from build123d import *

# Parameters (mm, degrees)
SWEEP1_PROFILE_R = 5


with BuildPart() as part:
    # Sweep1: sweep along a path in Sketch1
    with BuildLine(Plane.XY) as sweep1_path:
        Line((-60, 40), (-60, 10))
        ThreePointArc((-60, 10), (-57.071067812, 2.928932188), (-50, 0))
        Line((-50, 0), (50, 0))
        ThreePointArc((50, 0), (57.071067812, 2.928932188), (60, 10))
        Line((60, 10), (60, 40))
    # Sweep1 profile (on start of the path) → Sweep1 (sweep)
    with BuildSketch(Plane(origin=(-60, 40, 0), x_dir=(-1, 0, 0), z_dir=(0, -1, 0))):
        Circle(SWEEP1_PROFILE_R)
    sweep(path=sweep1_path.line)


solid = part.part
CAD build for the part. Positions are in the model's coordinates, mm. A direction names the side the tool comes from. Round coordinates to 2 decimals unless told otherwise and drop trailing zeros. Order: outer loops, then holes, each group sorted by start corner. A loop starts at its lowest first (then second) coordinate and runs counter-clockwise, first axis right, second up. Notation, with made-up numbers: (-1, 22.5) -> (26, 22.5) arc R31 cw to (26, 48.5) -> close; hole circle Ø4 at (86.5, 46.5). An arc over 180 degrees is marked (long way). Write item = value, one per line. Start each with the question number.
(1) Cut at B-B, the plane y = 31. List the corners of the cut face in (x, z), then the cut area to 3 significant figures.
(2) Pull direction X, two halves, no side cores. Call faces 3 (the cylindrical face through (-55, 25, 0)), 4 (the cylindrical face through (55, 25, 0)), 5 (the flat face through (-60, 40, 0)): released by +X, released by -X, zero draft, split by the parting line, or undercut.
(3) Probe line 1 (Y direction, x = 24.5, z = 0.5); line 2 (X direction, y = 35, z = 0.75); line 3 (X direction, y = 13, z = -2). List the from-to ranges inside material, lowest first. Write a range as [from, to].
(4) Pin check, flat tips, straight feed: P1, Ø5, axis at y = 11, z = -3.5, coming from the -X side; P2, Ø1, axis at y = 3, z = -2.5, coming from the -X side; P3, Ø1.5, axis at y = 7.5, z = -2.5, coming from the -X side. Stop position of each tip, or through.
(5) Cut at A-A, the plane z = 0. List the corners of the cut face in (x, y), then the cut area to 3 significant figures.
(6) Cut at C-C, the plane x = 40.5. List the corners of the cut face in (y, z).
(7) Which spindle directions (+Z, -Z, +X, -X, +Y, -Y) get a long thin tool onto all of the face, cutting with end or side? Do faces 1 (the cylindrical face through (0.7, 1.08, 4.88)), 2 (the flat face through (60, 40, 0)). Say none if no direction does.
Model answer:
q1.outline = circle Ø10 at (-60, 0); circle Ø10 at (60, 0)
q1.area = 157 mm2
q2.face_3 = undercut
q2.face_4 = undercut
q2.face_5 = zero draft
q3.line_1 = [-4.97, 4.97]
q3.line_2 = [-64.94, -55.06], [55.06, 64.94]
q3.line_3 = [-64.58, -55.42], [55.42, 64.58]
q4.P1 = -64.9
q4.P2 = -62.9
q4.P3 = -64.49
q5.outline = (-65, 10) arc R15 ccw to (-50, -5) -> (50, -5) arc R15 ccw to (65, 10) -> (65, 40) -> (55, 40) -> (55, 10) arc R5 cw to (50, 5) -> (-50, 5) arc R5 cw to (-55, 10) -> (-55, 40) -> (-65, 40) -> close
q5.area = 1,910 mm2
q6.outline = circle Ø10 at (0, 0)
q7.face_1 = none
q7.face_2 = +Z, -Z, +X, -X, +Y
